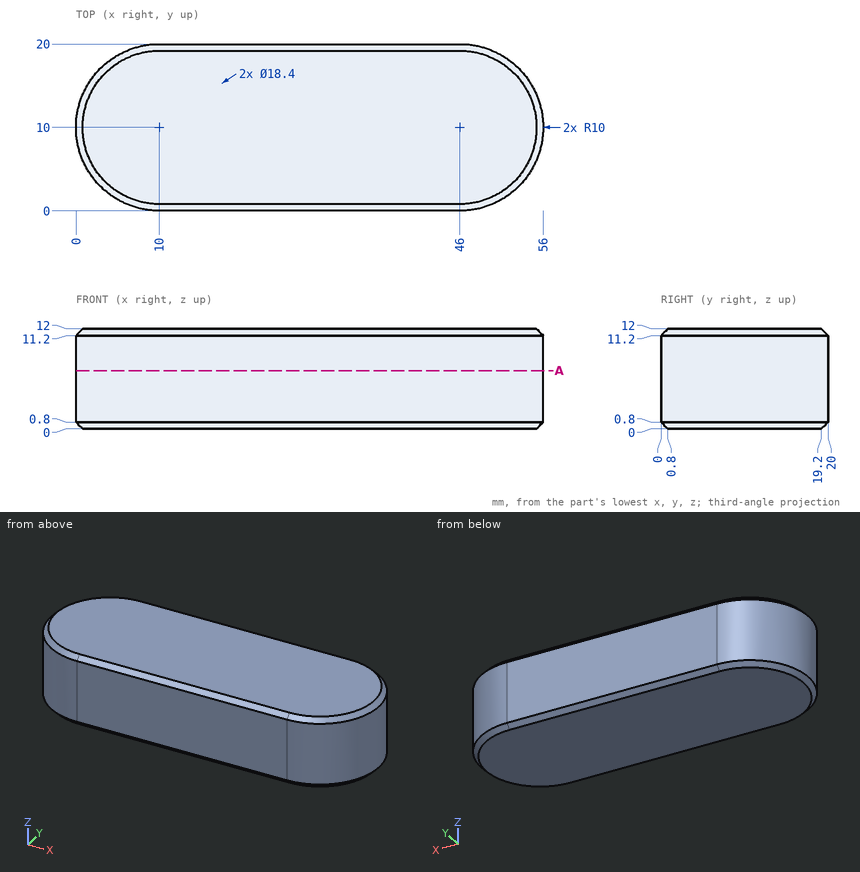
Here's the drawing with two shaded views (mm, measured from the low corner). I have some questions. Give positions to 0.01 mm unless a question says otherwise; leave off trailing zeros. Loops run counter-clockwise (first coordinate to the right, second up) from the corner with the lowest first, then second, coordinate; pieces in that order, holes last. Notation, with made-up numbers: (-26.75, 34.5) - (10.25, 34.5) arc R15 cw to (10.25, 59.5) - close; hole circle Ø1 at (31, 74). An arc over 180 degrees is marked (long way). Answer in a Markdown table with one row per item. Add a question column.
Q1. For pin 1 (3 mm diameter, centred on y = 14.5, z = 5.5, fed in from +X); pin 2 (1.5 mm diameter, centred on y = 12.5, z = 2, fed in from +X); pin 3 (6 mm diameter, centred on y = 17, z = 9.5, fed in from +X), each with a flat end and sliding along its axis, tell me the tip position at first contact or that it passes through.
Q2. Please list where these lines run through material, in increasing order: L1, parallel to X at y = 10.25, z = 1; L2, parallel to X at y = 7.25, z = 0.5; L3, parallel to Y at x = 20, z = 11.5. Write a range as from..to.
Q3. If we section it at A-A (z = 7): List the corners of the cut face in (x, y) for me.
The answers:
| question | item | result |
|---|---|---|
| 1 | pin 1 | stops at x = 55.54 |
| 1 | pin 2 | stops at x = 55.85 |
| 1 | pin 3 | stops at x = 55.17 |
| 2 | L1 | x = 0..56 |
| 2 | L2 | x = 0.7..55.3 |
| 2 | L3 | y = 0.3..19.7 |
| 3 | outline | (10, 0) - (46, 0) arc R10 ccw to (46, 20) - (10, 20) arc R10 ccw to start |
